Geometry check sheet. Reference: the model listing, model coordinates, mm. A direction names the side the tool comes from. Round coordinates to 2 decimals unless told otherwise and drop trailing zeros. Loops run counter-clockwise (first coordinate to the right, second up) from the corner with the lowest first, then second, coordinate; pieces in that order, holes last.
```python
from build123d import *

# Parameters (mm, degrees)
SKETCH1_R               = 8
SKETCH1_R_2             = 3
SKETCH3_R               = 3
BOSS_EXTRUDE1_DEPTH     = 3
CUT_EXTRUDE2_DEPTH      = 731.265705073
CUT_EXTRUDE2_DEPTH_BACK = 731.265705073
SKETCH4_R               = 2.5


with BuildPart() as part:
    # Sweep1: sweep along a path in Sketch2
    with BuildLine(Plane(origin=(0, 0, 0), x_dir=(0, 0, -1), z_dir=(1, 0, 0))) as sweep1_path:
        Line((0, 0), (-0.05, 0))
        ThreePointArc((-0.05, 0), (-7.085712473, -2.914287527), (-10, -9.95))
        Line((-10, -9.95), (-10, -730))
    # Sketch1 → Sweep1 (sweep)
    with BuildSketch(Plane.XY):
        Circle(SKETCH1_R)
        Circle(SKETCH1_R_2, mode=Mode.SUBTRACT)
    sweep(path=sweep1_path.line)

    # Sketch3 → Boss-Extrude1 (add)
    with BuildSketch(Plane.XZ.offset(730)):
        with Locations(Location((0, 10, 0), (0, 0, 270))):
            Circle(SKETCH3_R)
    extrude(amount=-BOSS_EXTRUDE1_DEPTH)

    # Sketch4 → Cut-Extrude2 (cut, two sides: drawn at the far end of the back side and taken through both)
    with BuildSketch(Plane.XY.offset(-CUT_EXTRUDE2_DEPTH_BACK)):
        with Locations((0, -724.5)):
            Circle(SKETCH4_R)
    extrude(amount=CUT_EXTRUDE2_DEPTH + CUT_EXTRUDE2_DEPTH_BACK, mode=Mode.SUBTRACT)


solid = part.part
```
1) Gauge pin test, flat ends, axial feed: pin 1 (2 mm diameter, centred on y = -216.5, z = 15.5, fed in from +X); pin 2 (4.5 mm diameter, centred on x = 0, y = -724.5, fed in from -Z) (3 decimals); pin 3 (8 mm diameter, centred on x = 0, y = 0, fed in from +Z); pin 4 (1.8 mm diameter, centred on x = -1.5, z = 9.5, fed in from +Y). Record the tip position at first contact, or that the pin passes through.
Report:
pin 1: stops at x = 6.61
pin 2: passes through
pin 3: stops at z = 16.99
pin 4: stops at y = 5.7
2) Access from +Z, -Z, +X, -X, +Y, -Y to the whole of each face (thin tool, end or side, straight path). Record for faces 1 (the face through (3.4, 0.1, 0)), 2 (the face through (-1.73, -375.02, 2.19)).
Report:
face 1: -Z, +X, -X, +Y, -Y
face 2: -Y
3) Sectioned sample at A-A, the plane y = -539. Record the cut outline in (x, z), then the cut area to 3 significant figures.
Report:
outline: circle Ø16 at (0, 10); hole circle Ø6 at (0, 10)
area: 173 mm2
4) Scan lines: line 1 along X through (y, z) = (-265, 10.25); line 2 along Z through (x, y) = (0.5, -343.5); line 3 along Y through (x, z) = (2, 9). Record each from-to range of solid material in increasing order.
Report:
line 1: x = -8 to -2.99, 2.99 to 8
line 2: z = 2.02 to 7.04, 12.96 to 17.98
line 3: y = -730 to -727, -1.68 to 5.32
